Input: part model. Units: mm. Frame: model coordinates. A direction names the side the tool comes from. Give positions to 0.01 mm unless a question says otherwise; leave off trailing zeros. Loops run counter-clockwise (first coordinate to the right, second up) from the corner with the lowest first, then second, coordinate; pieces in that order, holes last. Notation, with made-up numbers: (6.25, -13) -> (32.25, -13) arc R14 ccw to (32.25, -6) -> close; hole circle Ø10 at (1.25, 69.5). An arc over 180 degrees is marked (long way). One line per question, with ' | ' between items.
from build123d import *

# Parameters (mm, degrees)
BOSS_EXTRUDE1_DEPTH                    = 250
CBORE_FOR_M2_HEX_CAP_SCREW1_AT_2_COUNT = 2
CBORE_FOR_M2_HEX_CAP_SCREW1_AT_2_PITCH = 230
SKETCH_5_3_W                           = 5
SKETCH_5_3_H                           = 5
BOSS_EXTRUDE2_DEPTH                    = 1.2
SKETCH_5_3_2_W                         = 5
SKETCH_5_3_2_H                         = 5
BOSS_EXTRUDE3_DEPTH                    = 251.2
CUT_EXTRUDE1_START                     = -10
SKETCH6_R                              = 1.2
CUT_EXTRUDE1_DEPTH                     = 10


with BuildPart() as part:
    # Sketch1 → Boss-Extrude1 (new body)
    with BuildSketch(Plane(origin=(0, 0, 0), x_dir=(1, 0, 0), z_dir=(0, 1, 0))):
        Polygon((0, 0), (0, 20), (20, 20), (20, 0), (15, 0), (15, 5), (18, 5), (18, 8), (2, 8), (2, 5), (5, 5), (5, 0), align=None)
    extrude(amount=BOSS_EXTRUDE1_DEPTH)

    # Sketch4 → CBORE for M2 Hex Cap Screw1 (revolve, cut)
    with BuildSketch(Plane(origin=(0, 10, -15), x_dir=(0, 0, 1), z_dir=(0, 1, 0))):
        Polygon((0, 0), (0, 25.721032743), (1.2, 25), (1.2, 1.4), (3.8095, 1.4), (3.8095, 0.025), (3.8345, 0), align=None)
    cbore_for_m2_hex_cap_screw1 = revolve(axis=Axis((-6.35, 10, -15), (1, 0, 0)), mode=Mode.SUBTRACT)

    # CBORE for M2 Hex Cap Screw1 at 2: CBORE for M2 Hex Cap Screw1 ×2
    with Locations(*[(0, i * CBORE_FOR_M2_HEX_CAP_SCREW1_AT_2_PITCH, 0) for i in range(1, CBORE_FOR_M2_HEX_CAP_SCREW1_AT_2_COUNT)]):
        add(cbore_for_m2_hex_cap_screw1, mode=Mode.SUBTRACT)

    # Sketch 5_3 → Boss-Extrude2 (add)
    with BuildSketch(Plane(origin=(0, 250, 0), x_dir=(1, 0, 0), z_dir=(0, 1, 0))):
        with Locations((10, 15)):
            Rectangle(SKETCH_5_3_W, SKETCH_5_3_H)
    extrude(amount=BOSS_EXTRUDE2_DEPTH)

    # Sketch 5_3 2 → Boss-Extrude3 (add)
    with BuildSketch(Plane(origin=(0, 250, 0), x_dir=(1, 0, 0), z_dir=(0, 1, 0))):
        with Locations((10, 15)):
            Rectangle(SKETCH_5_3_2_W, SKETCH_5_3_2_H)
    extrude(amount=-BOSS_EXTRUDE3_DEPTH)

    # Sketch6 → Cut-Extrude1 (cut)
    with BuildSketch(Plane(origin=(12.5, 0, 0), x_dir=(0, 0, -1), z_dir=(1, 0, 0)).offset(CUT_EXTRUDE1_START)):
        with Locations(Location((15, 240, 0), (0, 0, 180))):
            Circle(SKETCH6_R)
        with Locations(Location((15, 10, 0), (0, 0, 180))):
            Circle(SKETCH6_R)
    extrude(amount=CUT_EXTRUDE1_DEPTH, mode=Mode.SUBTRACT)


solid = part.part
1. Reachability of faces 4 (the flat face through (10, 123, -8)), 5 (the flat face through (5, 123, -3)), 6 (the cylindrical face through (0.703, 236.223, -15.496)), 7 (the flat face through (0, 123, -10)), 8 (the flat face through (10, -1.2, -15)) from +Z, -Z, +X, -X, +Y, -Y: full face, straight path, thin tool, end or side. Return the list, or none.
Determined:
face 4: +Y, -Y | face 5: +Z, +Y, -Y | face 6: -X | face 7: +Z, -Z, -X, +Y, -Y | face 8: +Z, -Z, +X, -X, -Y
2. Pin query (flat end, axial travel): P1, Ø1, axis at x = 12.5, y = 145.5, coming from the +Z side; P2, Ø0.6, axis at y = -0.5, z = -14, coming from the +X side; P3, Ø6, axis at x = 6.5, z = -8.5, coming from the +Y side. Return the tip coordinate at first contact, or that it passes through.
Determined:
P1: stops at z = -8 | P2: stops at x = 12.5 | P3: stops at y = 250
3. Ray query, line 1 along Y through (x, z) = (0.85, -15); line 2 along Y through (x, z) = (8.75, -15); line 3 along Z through (x, y) = (16, 10). Return the intervals inside material, ascending. Write a range as from..to.
Determined:
line 1: y = 0..6.19, 13.81..236.19, 243.81..250 | line 2: y = -1.2..8.8, 11.2..238.8, 241.2..251.2 | line 3: z = -20..-16.2, -13.8..-8, -5..0
4. Pull-direction query (Z, two-part tool) for faces 1 (the cylindrical face through (0.7, 6.79, -12.95)), 2 (the flat face through (18, 123, 0)), 3 (the flat face through (10, 250, -12)); classes: pulls with the +Z half, pulls with the -Z half, needs draft (parallel to the pull), parting line crosses it, or undercut.
Determined:
face 1: undercut | face 2: pulls with the +Z half | face 3: needs draft
5. Section query A-A (y = 121). Output: boundary loops of the cut face in (x, z), then the cut area to 3 significant figures.
Determined:
outline: (0, -20) -> (20, -20) -> (20, 0) -> (15, 0) -> (15, -5) -> (18, -5) -> (18, -8) -> (2, -8) -> (2, -5) -> (5, -5) -> (5, 0) -> (0, 0) -> close | area: 302 mm2
